Source: CAD feature listing. Evaluate the final solid. Frame: model axes, mm. Face numbers are marked on the shaded views. A direction names the side the tool comes from. Coordinates: 2 decimals unless noted, no trailing zeros. Loops run counter-clockwise (first coordinate to the right, second up) from the corner with the lowest first, then second, coordinate; pieces in that order, holes last.
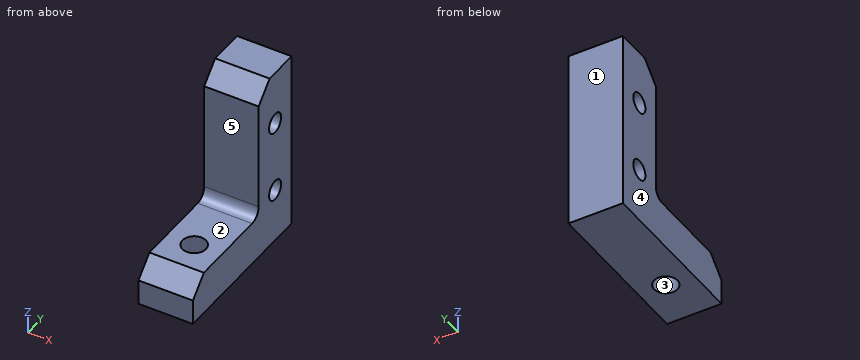
from build123d import *

# Parameters (mm, degrees)
SKETCH_1_W              = 15
SKETCH_1_H              = 15
EXTRUDE_1_DEPTH         = 25
SKETCH_2_W              = 15
SKETCH_2_H              = 30
EXTRUDE_2_DEPTH         = 12
HOLE_WIZARD_6_5_6_5_1_D = 6.5
FILLET_1_R              = 3
CHAMFER_2_SIZE          = 5
HOLE_WIZARD_5_5_5_5_1_D = 5.5


with BuildPart() as part:
    # 草图1 → 凸台-拉伸1 (new, symmetric)
    with BuildSketch(Plane.XY):
        Rectangle(SKETCH_1_W, SKETCH_1_H)
    extrude(amount=EXTRUDE_1_DEPTH, both=True)

    # 草图2 → 凸台-拉伸2 (add)
    with BuildSketch(Plane(origin=(0, 0, -25), x_dir=(-1, 0, 0), z_dir=(0, 0, -1))):
        with Locations((0, -22.5)):
            Rectangle(SKETCH_2_W, SKETCH_2_H)
    extrude(amount=-EXTRUDE_2_DEPTH)

    # Ø6.5 (6.5) 直径孔1 (through all)
    with Locations(Plane.XY.offset(-13)):
        with Locations((0, -24.5)):
            Hole(HOLE_WIZARD_6_5_6_5_1_D / 2)

    # 圆角1
    fillet_1_edges = [part.edges().sort_by_distance(p)[0] for p in [
        (0, -7.5, -13),
    ]]
    fillet(fillet_1_edges, radius=FILLET_1_R)

    # 倒角2
    chamfer_2_edges = [part.edges().sort_by_distance(p)[0] for p in [
        (0, -37.5, -13),
        (0, -7.5, 25),
    ]]
    chamfer(chamfer_2_edges, length=CHAMFER_2_SIZE)

    # Ø5.5 (5.5) 直径孔1 (through all)
    with Locations(Plane(origin=(7.5, 0, 0), x_dir=(0, 0, -1), z_dir=(1, 0, 0))):
        with Locations((10, 0), (-10, 0)):
            Hole(HOLE_WIZARD_5_5_5_5_1_D / 2)


solid = part.part
Q1. Contact query for flat-ended pins moving along their axis: pin 1 Ø5 at (y, z) = (0, -10) entering from +X; pin 2 Ø7.5 at (x, y) = (1.5, -26) entering from +Z; pin 3 Ø3 at (x, z) = (2, 9.5) entering from -Y; pin 4 Ø4 at (x, y) = (0, -11.5) entering from +Z. Output: stop coordinate, or through.
Q2. Access query for the marked faces 1 and 2. Directions: +Z, -Z, +X, -X, +Y, -Y. A direction counts if a zero-diameter tool reaches every point of the face in a straight line with its end or side. Return the directions, or none.
Q3. Section A-A, the plane x = 0. Return the cut outline in (y, z).
Q4. Section D-D, the plane y = 0. Return the cut outline in (x, z), plus the area to 3 significant figures.
Q5. Line query: line 1 along Y through (x, z) = (1, -10); line 2 along Z through (x, y) = (-4.25, -1); line 3 along Z through (x, y) = (-6.5, -2). Output: solid intervals per line, ascending.
Q6. Section B-B, the plane z = 10. Return the cut outline in (x, y).
Q7. Draft query along Y for the marked faces 3, 4 and 5. Return one class per face: +Y half, -Y half, draft (parallel to the pull), parting line (faces both ways), or undercut.
Q8. Section C-C, the plane y = -24.5. Return the cut outline in (x, z), plus the area to 3 significant figures.
Derived:
1. pin 1: passes through
1. pin 2: stops at z = -13
1. pin 3: stops at y = -7.5
1. pin 4: stops at z = -12.83
2. face 1: +Z, -Z, +X, -X, +Y
2. face 2: +Z, +X, -X, -Y
3. outline: (-37.5, -25) - (-27.75, -25) - (-27.75, -13) - (-32.5, -13) - (-37.5, -18) - close; (-21.25, -25) - (7.5, -25) - (7.5, 25) - (-2.5, 25) - (-7.5, 20) - (-7.5, -10) arc R3 cw to (-10.5, -13) - (-21.25, -13) - close; hole circle Ø5.5 at (0, -10); hole circle Ø5.5 at (0, 10)
4. outline: (-7.5, -25) - (7.5, -25) - (7.5, -12.75) - (-7.5, -12.75) - close; (-7.5, -7.25) - (7.5, -7.25) - (7.5, 7.25) - (-7.5, 7.25) - close; (-7.5, 12.75) - (7.5, 12.75) - (7.5, 25) - (-7.5, 25) - close
4. area: 585 mm2
5. line 1: y = -7.5 to -2.75, 2.75 to 7.5
5. line 2: z = -25 to -12.56, -7.44 to 7.44, 12.56 to 25
5. line 3: z = -25 to -11.89, -8.11 to 8.11, 11.89 to 25
6. outline: (-7.5, -7.5) - (7.5, -7.5) - (7.5, -2.75) - (-7.5, -2.75) - close; (-7.5, 2.75) - (7.5, 2.75) - (7.5, 7.5) - (-7.5, 7.5) - close
7. face 3: undercut
7. face 4: draft
7. face 5: -Y half
8. outline: (-7.5, -25) - (-3.25, -25) - (-3.25, -13) - (-7.5, -13) - close; (3.25, -25) - (7.5, -25) - (7.5, -13) - (3.25, -13) - close
8. area: 102 mm2
